Here's how the part is built. I have some questions about the finished solid (model axes, mm). A direction names the side the tool comes from. Round coordinates to 2 decimals unless told otherwise and drop trailing zeros. Loops run counter-clockwise (first coordinate to the right, second up) from the corner with the lowest first, then second, coordinate; pieces in that order, holes last. Notation, with made-up numbers: M 57.25,72.5 L 113.25,72.5 A15 ccw 113.25,77.5 Z; hole C 79,32 d7. An arc over 180 degrees is marked long. Answer as a JSON object with one key per item and string values.
from build123d import *

# Parameters (mm, degrees)
SKETCH1_R                      = 7
BOSS_EXTRUDE1_DEPTH            = 15
CUT_EXTRUDE1_START             = -1
SKETCH2_R                      = 7
SKETCH2_R_2                    = 6.25
CUT_EXTRUDE1_DEPTH             = 1
F_9_5_9_5_DIAMETER_HOLE1_D     = 9.5
F_9_5_9_5_DIAMETER_HOLE1_DEPTH = 11
F_9_5_9_5_DIAMETER_HOLE1_TIP   = 2.85408794
SKETCH4_R                      = 6.2
CUT_EXTRUDE2_DEPTH             = 5
CUT_EXTRUDE2_DRAFT             = -20
SKETCH5_R                      = 1.5
CUT_EXTRUDE3_DEPTH             = 10


with BuildPart() as part:
    # Sketch1 → Boss-Extrude1 (new body)
    with BuildSketch(Plane.XY):
        Circle(SKETCH1_R)
    extrude(amount=BOSS_EXTRUDE1_DEPTH)

    # Sketch2 → Cut-Extrude1 (cut)
    with BuildSketch(Plane.XY.offset(15).offset(CUT_EXTRUDE1_START)):
        Circle(SKETCH2_R)
        Circle(SKETCH2_R_2, mode=Mode.SUBTRACT)
    extrude(amount=CUT_EXTRUDE1_DEPTH, mode=Mode.SUBTRACT)

    # Ø9.5 (9.5) Diameter Hole1
    with Locations(Plane(origin=(0, 0, 0), x_dir=(-1, 0, 0), z_dir=(0, 0, -1))):
        with Locations((0, 0)):
            Hole(F_9_5_9_5_DIAMETER_HOLE1_D / 2, depth=F_9_5_9_5_DIAMETER_HOLE1_DEPTH)
            with Locations((0, 0, -(F_9_5_9_5_DIAMETER_HOLE1_DEPTH + F_9_5_9_5_DIAMETER_HOLE1_TIP / 2))):  # 118° drill point
                Cone(0, F_9_5_9_5_DIAMETER_HOLE1_D / 2, F_9_5_9_5_DIAMETER_HOLE1_TIP, mode=Mode.SUBTRACT)


with BuildPart() as cut_extrude2_tool:
    # Sketch4 → Cut-Extrude2 (with draft: the straight prism first)
    with BuildSketch(Plane(origin=(0, 0, 0), x_dir=(-1, 0, 0), z_dir=(0, 0, -1))):
        Circle(SKETCH4_R)
    extrude(amount=-CUT_EXTRUDE2_DEPTH)
    # Cut-Extrude2: the draft: its side faces are tilted about the plane it starts from
    cut_extrude2_sides = [cut_extrude2_tool.faces().sort_by_distance(p)[0] for p in [
        (6.2, 0, 2.5),
    ]]
    draft(cut_extrude2_sides, Plane(origin=(0, 0, 0), x_dir=(-1, 0, 0), z_dir=(0, 0, -1)), CUT_EXTRUDE2_DRAFT)


with BuildPart() as part_1:
    add(part.part)

    # Cut-Extrude2: cut by cut_extrude2_tool
    add(cut_extrude2_tool.part, mode=Mode.SUBTRACT)

    # Sketch5 → Cut-Extrude3 (cut, symmetric)
    with BuildSketch(Plane(origin=(0, 0, 0), x_dir=(1, 0, 0), z_dir=(0, 1, 0))):
        with Locations(Location((0, -7, 0), (0, 0, 270))):
            Circle(SKETCH5_R)
    extrude(amount=CUT_EXTRUDE3_DEPTH, both=True, mode=Mode.SUBTRACT)


solid = part_1.part
Item 1: On a 3-axis mill with a long thin cutter (end or side, diameter ignored), from which of +Z, -Z, +X, -X, +Y, -Y can I reach the whole of each face in a straight line? I mean faces 1 (the face through (0.179, -0.805, 13.358)), 2 (the face through (-3, 6, 14)). Say none if no direction works.
Resolved:
{"face 1": "-Z", "face 2": "+Z"}
Item 2: I want a section at C-C, the plane z = 2.25. Please give me the cut outline in (x, y).
Resolved:
{"outline": "C 0,0 d14; hole C 0,0 d10.76"}
Item 3: I want a section at A-A, the plane z = 7. Please give me the cut outline in (x, y), then the cut area to 3 significant figures.
Resolved:
{"outline": "M -1.5,-6.84 L -1.5,-4.51 A4.75 cw -1.5,4.51 L -1.5,6.84 A7 ccw Z; M 1.5,-6.84 A7 ccw 1.5,6.84 L 1.5,4.51 A4.75 cw 1.5,-4.51 Z", "area": "69.4 mm²"}
Item 4: Please list where these lines run through material, in increasing order: probe 1 along Y at (x, z) = (0, 9); probe 2 along X at (y, z) = (-4.75, 6.75); probe 3 along Y at (x, z) = (-1.5, 8.75). Write a range as from..to.
Resolved:
{"probe 1": "-7..-4.75, 4.75..7", "probe 2": "-5.14..-1.48, 1.48..5.14", "probe 3": "-6.84..-4.51, 4.51..6.84"}
Item 5: I'm going to push flat-ended pins straight in: pin 1 Ø1.5 at (y, z) = (3, 12) entering from -X; pin 2 Ø1 at (x, z) = (-4.5, 6.5) entering from +Y. Where does each tip first touch, or does it pass through?
Resolved:
{"pin 1": "x = -6.63", "pin 2": "y = 5.74"}
Item 6: I want a section at B-B, the plane x = 0.5. State how many separate pieces and enclosed holes the cut face has, then the cut area to 3 significant figures.
Resolved:
{"separate pieces": "3", "enclosed holes": "0", "area": "72.4 mm²"}
Item 7: I want a section at D-D, the plane z = 12.5. Please give me the cut outline in (x, y).
Resolved:
{"outline": "C 0,0 d14; hole C 0,0 d4.51"}
Item 8: If we mould it in two halves opening along Y, with no side actions, what happens to faces 3 (the face through (5.96, 1.88, 14.49)), 4 (the face through (0, 0, 15)), 5 (the face through (4.388, -1.819, 7.541))? For each: pulls with the +Y half, pulls with the -Y half, needs draft (parallel to the pull), parting line crosses it, or undercut.
Resolved:
{"face 3": "parting line crosses it", "face 4": "needs draft", "face 5": "undercut"}
